The model under review builds one solid part; all positions refer to its coordinate system, in mm. A direction names the side the tool comes from. Give positions to 0.01 mm unless a question says otherwise; leave off trailing zeros. Write each loop counter-clockwise with the first axis right and the second up, starting at its lowest first coordinate (ties: lowest second). Pieces come first, ordered by that corner, then holes. Notation, with made-up numbers: (84, -38.75) - (138, -38.75) arc R17 cw to (138, -14.75) - close; hole circle Ø4 at (64, 3.5). An arc over 180 degrees is marked (long way). One line per question, with ' | ' between items. Start each with the question number.
```python
from build123d import *

# Parameters (mm, degrees)
SKETCH_1_R          = 10.95
EXTRUDE_1_DEPTH     = 5
SKETCH_2_R          = 7.9
EXTRUDE_2_DEPTH     = 17
CUT_EXTRUDE_1_DEPTH = 5


with BuildPart() as part:
    # 草图1 → 凸台-拉伸1 (new body)
    with BuildSketch(Plane.XY):
        Circle(SKETCH_1_R)
    extrude(amount=EXTRUDE_1_DEPTH)

    # 草图2 → 凸台-拉伸2 (add)
    with BuildSketch(Plane(origin=(0, 0, 0), x_dir=(-1, 0, 0), z_dir=(0, 0, -1))):
        Circle(SKETCH_2_R)
    extrude(amount=-EXTRUDE_2_DEPTH)

    # 草图3 → 切除-拉伸1 (cut)
    with BuildSketch(Plane(origin=(0, 0, 0), x_dir=(-1, 0, 0), z_dir=(0, 0, -1))):
        Polygon((0, 4.734272207), (-4.1, 2.367136104), (-4.1, -2.367136104), (0, -4.734272207), (4.1, -2.367136104), (4.1, 2.367136104), align=None)
    extrude(amount=-CUT_EXTRUDE_1_DEPTH, mode=Mode.SUBTRACT)


solid = part.part
```
Item 1: Take a section at C-C (x = -2). Give the boundary of the cut face in (y, z), plus the area to 3 significant figures.
Item 2: Machinability: for faces 1 (the cylindrical face through (6.269, -4.807, 10.916)), 2 (the flat face through (-2.079, 3.534, 2.465)), 3 (the flat face through (0, 0, 17)), which of the approach directions +Z, -Z, +X, -X, +Y, -Y give a long, thin tool a straight path to every point of the face, cutting with its end or side? Answer none if there is none.
Item 3: Take a section at B-B (y = 0). Give the boundary of the cut face in (x, z), plus the area to 3 significant figures.
Item 4: For probe 1 along Z at (x, y) = (-3.25, 9.5); probe 2 along Y at (x, z) = (6.75, 7.25); probe 3 along X at (y, z) = (7.5, 1), list the stretches that pass through material, from the lowest coordinate up.
Item 5: Clearance check with flat-ended pins moving along their axes: P1, Ø3, axis at x = 3.5, y = -7.5, coming from the +Z side; P2, Ø2, axis at x = -2, y = 0, coming from the -Z side; P3, Ø2, axis at x = -2, z = 15.5, coming from the -Y side; P4, Ø2, axis at y = 4.5, z = 7.5, coming from the -X side. State where each tip first meets the part, or that it passes through.
Item 6: Take a section at D-D (z = 11). Give the boundary of the cut face in (x, y).
Item 7: The part is to be moulded in two halves that separate along X. For faces 4 (the flat face through (-5, 0, 0)), 5 (the flat face through (0, 0, 5)), 6 (the cylindrical face through (-8.69, -6.66, 2.46)), 7 (the flat face through (2.02, 3.57, 2.46)), say which applies: +X half, -X half, draft (parallel to the pull), parting line (faces both ways), or undercut.
Item 8: Take a section at A-A (z = 4.25). Give the boundary of the cut face in (x, y), plus the area to 3 significant figures.
Check sheet entries:
1) outline: (-10.77, 0) - (-3.58, 0) - (-3.58, 5) - (3.58, 5) - (3.58, 0) - (10.77, 0) - (10.77, 5) - (7.64, 5) - (7.64, 17) - (-7.64, 17) - (-7.64, 5) - (-10.77, 5) - close | area: 255 mm^2
2) face 1: +Z | face 2: -Z | face 3: +Z, +X, -X, +Y, -Y
3) outline: (-10.95, 0) - (-4.1, 0) - (-4.1, 5) - (4.1, 5) - (4.1, 0) - (10.95, 0) - (10.95, 5) - (7.9, 5) - (7.9, 17) - (-7.9, 17) - (-7.9, 5) - (-10.95, 5) - close | area: 258 mm^2
4) probe 1: z = 0 to 5 | probe 2: y = -4.1 to 4.1 | probe 3: x = -7.98 to 7.98
5) P1: stops at z = 17 | P2: stops at z = 5 | P3: stops at y = -7.84 | P4: stops at x = -7.08
6) outline: circle Ø15.8 at (0, 0)
7) face 4: draft | face 5: undercut | face 6: parting line | face 7: undercut
8) outline: circle Ø21.9 at (0, 0); hole (-4.1, -2.37) - (0, -4.73) - (4.1, -2.37) - (4.1, 2.37) - (0, 4.73) - (-4.1, 2.37) - close | area: 318 mm^2
